The model under review builds one solid part; all positions refer to its coordinate system, in mm. Round coordinates to 2 decimals unless told otherwise and drop trailing zeros. Loops run counter-clockwise (first coordinate to the right, second up) from the corner with the lowest first, then second, coordinate; pieces in that order, holes last. Notation, with made-up numbers: (-4, -8.75) -> (6, -8.75) arc R25 ccw to (6, 18.25) -> close; hole circle Ø9 at (83, -1). An arc over 180 degrees is marked (long way). Use a Markdown table: item, result. Add a question column.
1) Consider section A-A on z = 0. Give the boundary of the cut face in (x, y), plus the area to 3 significant figures.
2) Consider section B-B on x = 30. Give the boundary of the cut face in (y, z), plus the area to 3 significant figures.
3) Mouldability with a two-part tool opening along X and no side actions: class faces 1 (the cylindrical face through (21.78, 0.99, 69.15)), 2 (the cylindrical face through (66, 1, 0)), 3 (the flat face through (-53.4, 2, -16.4)) as released by +X, released by -X, zero draft, split by the parting line, or undercut.
4) Insertion check: pin 1 (4 mm diameter, centred on x = 0, z = -62.5, fed in from -Y). The pin has a flat end and moves straight along its axis. Give the tip position at first contact, or say it passes through.
5) Wall thickness on probe 1 along X at (y, z) = (1.9, -3); probe 2 along X at (y, z) = (0.6, 62.5); probe 3 along Z at (x, y) = (26.5, 1.4): over which ranges is each line inside the solid? List them lowest first.
6) Consider section D-D on y = 0.85. Give the boundary of the cut face in (x, z).
7) Consider section C-C on x = 0. Give the boundary of the cut face in (y, z).
from build123d import *

# Parameters (mm, degrees)
SKETCH1_R           = 72.5
SKETCH1_R_2         = 55.5
BOSS_EXTRUDE1_DEPTH = 2
SKETCH2_R           = 3.5
CUT_EXTRUDE1_DEPTH  = 103.549987811
CIRPATTERN1_COUNT   = 4


with BuildPart() as part:
    # Sketch1 → Boss-Extrude1 (new body)
    with BuildSketch(Plane(origin=(0, 0, 0), x_dir=(1, 0, 0), z_dir=(0, 1, 0))):
        with Locations(Location((0, 0, 0), (0, 0, 270))):
            Circle(SKETCH1_R)
        with Locations(Location((0, 0, 0), (0, 0, 270))):
            Circle(SKETCH1_R_2, mode=Mode.SUBTRACT)
    extrude(amount=BOSS_EXTRUDE1_DEPTH)

    # Sketch2 → Cut-Extrude1 (cut, through all)
    with BuildSketch(Plane(origin=(0, 2, 0), x_dir=(1, 0, 0), z_dir=(0, 1, 0))):
        with Locations(Location((0, 62.5, 0), (0, 0, 270))):
            Circle(SKETCH2_R)
    cut_extrude1 = extrude(amount=-CUT_EXTRUDE1_DEPTH, mode=Mode.SUBTRACT)

    # CirPattern1: Cut-Extrude1 ×4 about axis
    cirpattern1_axis = Axis((0, 0, 0), (0, 1, 0))
    for i in range(1, CIRPATTERN1_COUNT):
        add(cut_extrude1.rotate(cirpattern1_axis, i * 360 / CIRPATTERN1_COUNT), mode=Mode.SUBTRACT)


solid = part.part
Result set:
| question | item | result |
|---|---|---|
| 1 | outline | (-72.5, 0) -> (-66, 0) -> (-66, 2) -> (-72.5, 2) -> close; (-59, 0) -> (-55.5, 0) -> (-55.5, 2) -> (-59, 2) -> close; (55.5, 0) -> (59, 0) -> (59, 2) -> (55.5, 2) -> close; (66, 0) -> (72.5, 0) -> (72.5, 2) -> (66, 2) -> close |
| 1 | area | 40.0 mm2 |
| 2 | outline | (0, -66) -> (2, -66) -> (2, -46.69) -> (0, -46.69) -> close; (0, 46.69) -> (2, 46.69) -> (2, 66) -> (0, 66) -> close |
| 2 | area | 77.2 mm2 |
| 3 | face 1 | split by the parting line |
| 3 | face 2 | undercut |
| 3 | face 3 | zero draft |
| 4 | pin 1 | through |
| 5 | probe 1 | -72.44 to -64.3, -60.7 to -55.42, 55.42 to 60.7, 64.3 to 72.44 |
| 5 | probe 2 | -36.74 to -3.5, 3.5 to 36.74 |
| 5 | probe 3 | -67.48 to -48.76, 48.76 to 67.48 |
| 6 | outline | circle Ø145 at (0, 0); hole circle Ø7 at (-62.5, 0); hole circle Ø111 at (0, 0); hole circle Ø7 at (0, -62.5); hole circle Ø7 at (0, 62.5); hole circle Ø7 at (62.5, 0) |
| 7 | outline | (0, -72.5) -> (2, -72.5) -> (2, -66) -> (0, -66) -> close; (0, -59) -> (2, -59) -> (2, -55.5) -> (0, -55.5) -> close; (0, 55.5) -> (2, 55.5) -> (2, 59) -> (0, 59) -> close; (0, 66) -> (2, 66) -> (2, 72.5) -> (0, 72.5) -> close |
